Read the model definition and answer for the solid it produces. Units are mm, in the model's axes. Round coordinates to 2 decimals unless told otherwise and drop trailing zeros. Write each loop counter-clockwise with the first axis right and the second up, starting at its lowest first coordinate (ties: lowest second). Pieces come first, ordered by that corner, then holes. Notation, with made-up numbers: (70, 12.5) -> (98, 12.5) arc R22 ccw to (98, 20.5) -> close; hole circle Ø9 at (8.25, 18). An arc over 180 degrees is marked (long way). Return JSON: item names as keys, results as strings. Group by question number.
(1) A cutting plane is placed at A-A on y = 155. Give the vertices of the cut face in (x, z), then the cut area to 3 significant figures.
(2) Given pin 1 (14.5 mm diameter, centred on x = -43.98, y = -24.94, fed in from -Z), flat-ended and moving along its own axis, determine where the tip first touches the part or whether it passes through.
(3) A cutting plane is placed at C-C on z = 15.5. State how many separate pieces and enclosed holes the cut face has, then the cut area to 3 significant figures.
(4) The mould has two halves that part along Y. Classify faces 1 (the flat face through (444, 173, 0)), 2 (the flat face through (444, -54.941, 16)), 3 (the cylindrical face through (-52.8, 373.2, 16.2)): released by +Y, released by -Y, zero draft, split by the parting line, or undercut.
(5) Straight lines are drawn through the part: line 1 (X direction, y = 282, z = 18); line 2 (X direction, y = 82, z = 29); line 3 (Y direction, x = 339, z = 14.5). For each, find the intervals that lie inside material, in ascending order.
(6) A cutting plane is placed at B-B on x = 75. Give the vertices of the cut face in (y, z).
(7) A cutting plane is placed at D-D on y = 257. Give the vertices of the cut face in (x, z), then the cut area to 3 significant figures.
```python
from build123d import *

# Parameters (mm, degrees)
SKETCH1_W           = 1050
SKETCH1_H           = 450
BOSS_EXTRUDE1_DEPTH = 32
SKETCH2_R           = 125
CUT_EXTRUDE1_DEPTH  = 32
SKETCH3_R           = 12
CUT_EXTRUDE2_DEPTH  = 32
SKETCH7_R           = 3
CUT_EXTRUDE3_DEPTH  = 32
CIRPATTERN1_COUNT   = 4


with BuildPart() as part:
    # Sketch1 → Boss-Extrude1 (new body)
    with BuildSketch(Plane.XY):
        with Locations((451.017205348, 170.059190469)):
            Rectangle(SKETCH1_W, SKETCH1_H)
    extrude(amount=BOSS_EXTRUDE1_DEPTH)

    # Sketch2 → Cut-Extrude1 (cut)
    with BuildSketch(Plane.XY.offset(32)):
        with Locations((181.017205348, 170.059190469)):
            Circle(SKETCH2_R)
        with Locations((721.017205348, 170.059190469)):
            Circle(SKETCH2_R)
    extrude(amount=-CUT_EXTRUDE1_DEPTH, mode=Mode.SUBTRACT)

    # Sketch3 → Cut-Extrude2 (cut)
    with BuildSketch(Plane.XY.offset(32)):
        with Locations((-43.982794652, 365.059190469)):
            Circle(SKETCH3_R)
        with Locations((-43.982794652, 235.059190469)):
            Circle(SKETCH3_R)
        with Locations((-43.982794652, 105.059190469)):
            Circle(SKETCH3_R)
        with Locations((-43.982794652, -24.940809531)):
            Circle(SKETCH3_R)
        with Locations(Location((946.017205348, -24.940809531, 0), (0, 0, 180))):
            Circle(SKETCH3_R)
        with Locations(Location((946.017205348, 105.059190469, 0), (0, 0, 180))):
            Circle(SKETCH3_R)
        with Locations(Location((946.017205348, 235.059190469, 0), (0, 0, 180))):
            Circle(SKETCH3_R)
        with Locations(Location((946.017205348, 365.059190469, 0), (0, 0, 180))):
            Circle(SKETCH3_R)
        with Locations((451.017205348, 365.059190469)):
            Circle(SKETCH3_R)
        with Locations((451.017205348, 235.059190469)):
            Circle(SKETCH3_R)
        with Locations((451.017205348, 105.059190469)):
            Circle(SKETCH3_R)
        with Locations((451.017205348, -24.940809531)):
            Circle(SKETCH3_R)
    extrude(amount=-CUT_EXTRUDE2_DEPTH, mode=Mode.SUBTRACT)

    # Sketch5 → M36 Tapped Hole1 (revolve, cut)
    with BuildSketch(Plane(origin=(36.017205348, 315.059190469, 32), x_dir=(0, -1, 0), z_dir=(1, 0, 0))):
        Polygon((0, 0), (0, 101.613769904), (16, 92), (16, 0), align=None)
    m36_tapped_hole1 = revolve(axis=Axis((36.017205348, 315.059190469, 38.35), (0, 0, -1)), mode=Mode.SUBTRACT)

    # Mirror1: M36 Tapped Hole1 across plane
    add(m36_tapped_hole1.mirror(Plane.ZY.offset(-451.017205348)), mode=Mode.SUBTRACT)

    # Sketch7 → Cut-Extrude3 (cut)
    with BuildSketch(Plane.XY.offset(32)):
        with Locations((-43.982794652, 170.059190469)):
            Circle(SKETCH7_R)
    cut_extrude3 = extrude(amount=-CUT_EXTRUDE3_DEPTH, mode=Mode.SUBTRACT)

    # Mirror2: Cut-Extrude3 across plane
    add(cut_extrude3.mirror(Plane.ZY.offset(-451.017205348)), mode=Mode.SUBTRACT)

    # CirPattern1: M36 Tapped Hole1 ×4 about axis
    cirpattern1_axis = Axis((181.017205348, 170.059190469, 0), (0, 0, 1))
    for i in range(1, CIRPATTERN1_COUNT):
        add(m36_tapped_hole1.rotate(cirpattern1_axis, i * 360 / CIRPATTERN1_COUNT), mode=Mode.SUBTRACT)

    # Mirror3: M36 Tapped Hole1 across plane
    add(m36_tapped_hole1.mirror(Plane.ZY.offset(-451.017205348)), mode=Mode.SUBTRACT)

    # Mirror3 copy 1 sketch → Mirror3 copy 1 (revolve, cut)
    with BuildSketch(Plane(origin=(866.017205348, 25.059190469, 32), x_dir=(-1, 0, 0), z_dir=(0, 1, 0))):
        Polygon((0, 0), (0, -101.613769904), (16, -92), (16, 0), align=None)
    revolve(axis=Axis((866.017205348, 25.059190469, 38.35), (0, 0, 1)), mode=Mode.SUBTRACT)

    # Mirror3 copy 2 sketch → Mirror3 copy 2 (revolve, cut)
    with BuildSketch(Plane(origin=(576.017205348, 25.059190469, 32), x_dir=(0, 1, 0), z_dir=(1, 0, 0))):
        Polygon((0, 0), (0, -101.613769904), (16, -92), (16, 0), align=None)
    revolve(axis=Axis((576.017205348, 25.059190469, 38.35), (0, 0, 1)), mode=Mode.SUBTRACT)

    # Mirror3 copy 3 sketch → Mirror3 copy 3 (revolve, cut)
    with BuildSketch(Plane(origin=(576.017205348, 315.059190469, 32), x_dir=(1, 0, 0), z_dir=(0, -1, 0))):
        Polygon((0, 0), (0, -101.613769904), (16, -92), (16, 0), align=None)
    revolve(axis=Axis((576.017205348, 315.059190469, 38.35), (0, 0, 1)), mode=Mode.SUBTRACT)


solid = part.part
```
Checks:
{
 "1": {"outline": "(-73.98, 0) -> (56.93, 0) -> (56.93, 32) -> (-73.98, 32) -> close; (305.11, 0) -> (596.93, 0) -> (596.93, 32) -> (305.11, 32) -> close; (845.11, 0) -> (976.02, 0) -> (976.02, 32) -> (845.11, 32) -> close", "area": "17,700 mm^2"},
 "2": {"pin 1": "passes through"},
 "3": {"separate pieces": "1", "enclosed holes": "24", "area": "362,000 mm^2"},
 "4": {"face 1": "zero draft", "face 2": "released by -Y", "face 3": "undercut"},
 "5": {"line 1": "x = -73.98 to 125.39, 236.64 to 665.39, 776.64 to 976.02", "line 2": "x = -73.98 to 92.3, 269.73 to 632.3, 809.73 to 976.02", "line 3": "y = -54.94 to 15.71, 34.41 to 305.71, 324.41 to 395.06"},
 "6": {"outline": "(-54.94, 0) -> (103.84, 0) -> (103.84, 32) -> (-54.94, 32) -> close; (236.28, 0) -> (395.06, 0) -> (395.06, 32) -> (236.28, 32) -> close"},
 "7": {"outline": "(-73.98, 0) -> (91.2, 0) -> (91.2, 32) -> (-73.98, 32) -> close; (270.83, 0) -> (631.2, 0) -> (631.2, 32) -> (270.83, 32) -> close; (810.83, 0) -> (976.02, 0) -> (976.02, 32) -> (810.83, 32) -> close", "area": "22,100 mm^2"}
}
